The model under review builds one solid part; all positions refer to its coordinate system, in mm. A direction names the side the tool comes from. Give positions to 0.01 mm unless a question says otherwise; leave off trailing zeros. Order: outer loops, then holes, each group sorted by start corner. A loop starts at its lowest first (then second) coordinate and runs counter-clockwise, first axis right, second up. Notation, with made-up numbers: M -25,-26 L -2,-26 A21 cw -2,-1 Z; hole C -37,24.25 d2. An arc over 180 degrees is marked long. One line per question, with ' | ' between items. Start each with the question number.
1. We need section D-D on x = 75. Write out the cut boundary in (y, z).
2. We need section C-C on y = 207. Write out the cut boundary in (x, z), then the cut area to 3 significant figures.
3. Insertion check: P1, Ø6.5, axis at x = 91, y = 141.5, coming from the -Z side; P2, Ø4, axis at x = 18.5, y = 120.5, coming from the -Z side; P3, Ø5.5, axis at x = 37, y = 230.5, coming from the +Z side. Each pin has a flat end and moves straight along its axis. Give the tip position at first contact, or say it passes through.
4. Wall thickness on L1, parallel to Y at x = 10, z = 4; L2, parallel to X at y = 230.5, z = 85; L3, parallel to Y at x = 81, z = 85.75: over which ranges is each line inside the solid? List them lowest first.
5. We need section A-A on y = 65. Write out the cut boundary in (x, z).
6. We need section B-B on x = 106. Write out the cut boundary in (y, z), then the cut area to 3 significant figures.
7. For faces 1 (the face through (96, 99, 57)), 2 (the face through (-52, 201, 88)), 3 (the face through (20, 211, 84)), 4 (the face through (92, 169, 48)), 5 (the face through (-56, 167, 106)), list the 3-axis set-ups (+Z, -Z, +X, -X, +Y, -Y) from which the entire face can be reached by the end or side of a thin tool; tool diameter is ignored.
8. The part is to be moulded in two halves that separate along X. For faces 6 (the face through (71, 260, 81)), 7 (the face through (33, 155, 80)), 8 (the face through (116, 40, 4)), say which applies: +X half, -X half, draft (parallel to the pull), parting line (faces both ways), or undercut.
```python
from build123d import *

# Parameters (mm, degrees)
SKETCH_1_W             = 116
SKETCH_1_H             = 80
EXTRUDE_1_DEPTH        = 8
SKETCH_2_W             = 8
SKETCH_2_H             = 80
EXTRUDE_2_DEPTH        = 80
SKETCH_4_W             = 8
SKETCH_4_H             = 40
EXTRUDE_3_DEPTH        = 180
SKETCH_5_W             = 60
SKETCH_5_H             = 8
EXTRUDE_4_DEPTH        = 80
SKETCH_8_W             = 8
SKETCH_8_H             = 40
EXTRUDE_7_DEPTH        = 30
SKETCH_10_W            = 40
SKETCH_10_H            = 8
EXTRUDE_8_DEPTH        = 80
SKETCH_11_W            = 8
SKETCH_11_H            = 40
EXTRUDE_9_DEPTH        = 150
SKETCH_12_W            = 8
SKETCH_12_H            = 93
EXTRUDE_10_DEPTH       = 68
SKETCH_14_W            = 8
SKETCH_14_H            = 93
EXTRUDE_12_DEPTH       = 42
FILLET_1_R             = 5
FILLET_2_R             = 5
HOLE_WIZARD_9_0_9_1_D  = 9
HOLE_WIZARD_M5_1_D     = 4.2
HOLE_WIZARD_M6_1_D     = 5
HOLE_WIZARD_M5_2_D     = 4.2
HOLE_WIZARD_M5_2_DEPTH = 10.4
HOLE_WIZARD_M5_2_TIP   = 1.2618073
EXTRUDE_15_DEPTH       = 8
FILLET_3_R             = 5


with BuildPart() as part:
    # 草图1 → 凸台-拉伸1 (new body)
    with BuildSketch(Plane.XY):
        with Locations((58, 40)):
            Rectangle(SKETCH_1_W, SKETCH_1_H)
    extrude(amount=EXTRUDE_1_DEPTH)

    # 草图2 → 凸台-拉伸2 (add)
    with BuildSketch(Plane.XY.offset(8)):
        with Locations((24, 40)):
            Rectangle(SKETCH_2_W, SKETCH_2_H)
        with Locations((92, 40)):
            Rectangle(SKETCH_2_W, SKETCH_2_H)
    extrude(amount=EXTRUDE_2_DEPTH)

    # 草图4 → 凸台-拉伸3 (add)
    with BuildSketch(Plane(origin=(0, 80, 0), x_dir=(1, 0, 0), z_dir=(0, 1, 0))):
        with Locations((92, -68)):
            Rectangle(SKETCH_4_W, SKETCH_4_H)
    extrude(amount=EXTRUDE_3_DEPTH)

    # 草图5 → 凸台-拉伸4 (add)
    with BuildSketch(Plane.XY.offset(8)):
        with Locations((58, 4)):
            Rectangle(SKETCH_5_W, SKETCH_5_H)
    extrude(amount=EXTRUDE_4_DEPTH)

    # 草图8 → 凸台-拉伸7 (add)
    with BuildSketch(Plane(origin=(0, 80, 0), x_dir=(1, 0, 0), z_dir=(0, 1, 0))):
        with Locations((24, -68)):
            Rectangle(SKETCH_8_W, SKETCH_8_H)
    extrude(amount=EXTRUDE_7_DEPTH)

    # 草图10 → 凸台-拉伸8 (add)
    with BuildSketch(Plane.ZY.offset(-20)):
        with Locations((68, 106)):
            Rectangle(SKETCH_10_W, SKETCH_10_H)
    extrude(amount=EXTRUDE_8_DEPTH)

    # 草图11 → 凸台-拉伸9 (add)
    with BuildSketch(Plane(origin=(0, 110, 0), x_dir=(1, 0, 0), z_dir=(0, 1, 0))):
        with Locations((-56, -68)):
            Rectangle(SKETCH_11_W, SKETCH_11_H)
    extrude(amount=EXTRUDE_9_DEPTH)

    # 草图12 → 凸台-拉伸10 (add)
    with BuildSketch(Plane.ZY.offset(-88)):
        with Locations((84, 213.5)):
            Rectangle(SKETCH_12_W, SKETCH_12_H)
    extrude(amount=EXTRUDE_10_DEPTH)

    # 草图14 → 凸台-拉伸12 (add)
    with BuildSketch(Plane.XY.offset(88)):
        with Locations((-56, 213.5)):
            Rectangle(SKETCH_14_W, SKETCH_14_H)
    extrude(amount=EXTRUDE_12_DEPTH)

    # 圆角1
    fillet_1_edges = [part.edges().sort_by_distance(p)[0] for p in [
        (-56, 260, 48),
        (24, 80, 48),
        (92, 80, 48),
        (92, 260, 48),
        (-56, 260, 130),
        (-56, 167, 130),
        (20, 260, 84),
    ]]
    fillet(fillet_1_edges, radius=FILLET_1_R)

    # 圆角2
    fillet_2_edges = [part.edges().sort_by_distance(p)[0] for p in [
        (0, 80, 4),
        (0, 0, 4),
        (116, 80, 4),
        (116, 0, 4),
    ]]
    fillet(fillet_2_edges, radius=FILLET_2_R)

    # Ø9.0 (9) 直径孔1 (through all)
    with Locations(Plane.XY.offset(8)):
        with Locations((106, 15), (106, 65)):
            hole_wizard_9_0_9_1 = Hole(HOLE_WIZARD_9_0_9_1_D / 2)

    # 镜向1: Ø9.0 (9) 直径孔1 across plane
    add(hole_wizard_9_0_9_1.mirror(Plane(origin=(58, 0, 0), x_dir=(0, 0, 1), z_dir=(1, 0, 0))), mode=Mode.SUBTRACT)

    # M5 螺纹孔1 (through all)
    with Locations(Plane.XY.offset(88)):
        with Locations((37, 196.5), (81, 196.5), (81, 230.5), (37, 230.5)):
            Hole(HOLE_WIZARD_M5_1_D / 2)

    # M6 螺纹孔1 (through all)
    with Locations(Plane(origin=(-52, 0, 0), x_dir=(0, 0, -1), z_dir=(1, 0, 0))):
        with Locations((-96, 252.5), (-122, 252.5), (-122, 174.5), (-96, 174.5)):
            Hole(HOLE_WIZARD_M6_1_D / 2)

    # M5 螺纹孔2
    with Locations(Plane(origin=(96, 0, 0), x_dir=(0, 0, -1), z_dir=(1, 0, 0))):
        with Locations((-72, 250), (-54, 250)):
            Hole(HOLE_WIZARD_M5_2_D / 2, depth=HOLE_WIZARD_M5_2_DEPTH)
            with Locations((0, 0, -(HOLE_WIZARD_M5_2_DEPTH + HOLE_WIZARD_M5_2_TIP / 2))):  # 118° drill point
                Cone(0, HOLE_WIZARD_M5_2_D / 2, HOLE_WIZARD_M5_2_TIP, mode=Mode.SUBTRACT)

    # 草图27 → 凸台-拉伸15 (add)
    with BuildSketch(Plane.XY.offset(88)):
        Polygon((88, 87), (88, 167), (20, 167), (20, 160), (-52, 160), (-52, 110), (28, 110), (28, 87), align=None)
    extrude(amount=-EXTRUDE_15_DEPTH)

    # 圆角3
    fillet_3_edges = [part.edges().sort_by_distance(p)[0] for p in [
        (20, 160, 84),
    ]]
    fillet(fillet_3_edges, radius=FILLET_3_R)


solid = part.part
```
Entries:
1) outline: M 0,0 L 80,0 L 80,8 L 8,8 L 8,88 L 0,88 Z; M 87,80 L 260,80 L 260,88 L 87,88 Z
2) outline: M -60,48 L -52,48 L -52,130 L -60,130 Z; M 20,80 L 88,80 L 88,48 L 96,48 L 96,88 L 20,88 Z | area: 1,520 mm^2
3) P1: stops at z = 48 | P2: stops at z = 80 | P3: stops at z = 88
4) L1: y = 0 to 10.5, 19.5 to 60.5, 69.5 to 80 | L2: x = -60 to -52, 20 to 34.9, 39.1 to 78.9, 83.1 to 96 | L3: y = 0 to 8, 87 to 194.4, 198.6 to 228.4, 232.6 to 260
5) outline: M 0,0 L 5.5,0 L 5.5,8 L 0,8 Z; M 14.5,0 L 101.5,0 L 101.5,8 L 96,8 L 96,88 L 88,88 L 88,8 L 28,8 L 28,88 L 20,88 L 20,8 L 14.5,8 Z; M 110.5,0 L 116,0 L 116,8 L 110.5,8 Z
6) outline: M 0,0 L 10.5,0 L 10.5,8 L 0,8 Z; M 19.5,0 L 60.5,0 L 60.5,8 L 19.5,8 Z; M 69.5,0 L 80,0 L 80,8 L 69.5,8 Z | area: 496 mm^2
7) face 1: +Z, +X, +Y, -Y | face 2: -Z, +Y | face 3: +Z, -Z, +Y | face 4: -Z, +X, -X, +Y | face 5: +Z, +X, -X, -Y
8) face 6: draft | face 7: undercut | face 8: +X half
